Read the model definition and answer for the solid it produces. Units are mm, in the model's axes. A direction names the side the tool comes from. Give positions to 0.01 mm unless a question says otherwise; leave off trailing zeros. Loops run counter-clockwise (first coordinate to the right, second up) from the corner with the lowest first, then second, coordinate; pieces in that order, holes last. Notation, with made-up numbers: (63.5, 80) - (105.5, 80) arc R10 cw to (105.5, 92) - close; hole circle Ø11 at (38, 66.5). An arc over 180 degrees is marked (long way). Write item = value, one per line.
```python
from build123d import *

# Parameters (mm, degrees)
BOSS_EXTRUDE1_DEPTH = 22.352


with BuildPart() as part:
    # Sketch1 → Boss-Extrude1 (new body)
    with BuildSketch(Plane.XY):
        with BuildLine():
            Line((0, 11.112), (22.35, 11.112))
            Line((22.35, 11.112), (22.35, 7.112))
            Line((22.35, 7.112), (0, 7.112))
            ThreePointArc((0, 7.112), (-5.028943428, 5.028943428), (-7.112, 0))
            ThreePointArc((-7.112, 0), (-8.951369414, -4.440630586), (-13.392, -6.28))
            Line((-13.392, -6.28), (-23.192, -6.28))
            Line((-23.192, -6.28), (-23.192, -2.28))
            Line((-23.192, -2.28), (-13.392, -2.28))
            ThreePointArc((-13.392, -2.28), (-11.779796539, -1.612203461), (-11.112, 0))
            ThreePointArc((-11.112, 0), (-7.857370553, 7.857370553), (0, 11.112))
        make_face()
    extrude(amount=BOSS_EXTRUDE1_DEPTH)


solid = part.part
```
1) A cutting plane is placed at C-C on y = -0.5. Determine the outline of the cut face in (x, z), then the cut area to 3 significant figures.
Output:
outline = (-11.17, 0) - (-7.13, 0) - (-7.13, 22.35) - (-11.17, 22.35) - close
area = 90.2 mm²
2) A tool of negligible diameter and unlimited length cuts with its end or side. For faces 1 (the face through (-23.192, -4, 11)), 2 (the face through (-18, -2.28, 11)), 3 (the face through (11, 7.112, 11)), from which of +Z, -Z, +X, -X, +Y, -Y can it reach the whole face along a straight path? Write none if from no direction.
Output:
face_1 = +Z, -Z, -X, +Y, -Y
face_2 = +Z, -Z, -X, +Y
face_3 = +Z, -Z, +X, -Y
3) A cutting plane is placed at B-B on x = 9.5. Determine the outline of the cut face in (y, z), then the cut area to 3 significant figures.
Output:
outline = (7.11, 0) - (11.11, 0) - (11.11, 22.35) - (7.11, 22.35) - close
area = 89.4 mm²
4) Each of these flat-tipped pins is pushed along its axis until it touches: P1, Ø1, axis at y = -1.5, z = 13.5, coming from the +X side; P2, Ø3, axis at x = 14, z = 11.5, coming from the -Y side; P3, Ø4, axis at y = -4, z = 5.5, coming from the +X side. Where does it stop, or does it pass through?
Output:
P1 = -7.19
P2 = 7.11
P3 = -7.44
5) Find the intervals of material crossed by probe 1 along Y at (x, z) = (-18, 20.5); probe 2 along Y at (x, z) = (13.5, 15); probe 3 along X at (y, z) = (-5.5, 8), in increasing order.
Output:
probe_1 = -6.28 to -2.28
probe_2 = 7.11 to 11.11
probe_3 = -23.19 to -10.36
6) A cutting plane is placed at A-A on z = 16.5. Determine the outline of the cut face in (x, y), then the cut area to 3 significant figures.
Output:
outline = (-23.19, -6.28) - (-13.39, -6.28) arc R6.28 ccw to (-7.11, 0) arc R7.11 cw to (0, 7.11) - (22.35, 7.11) - (22.35, 11.11) - (0, 11.11) arc R11.11 ccw to (-11.11, 0) arc R2.28 cw to (-13.39, -2.28) - (-23.19, -2.28) - close
area = 213 mm²
